from build123d import *

# Parameters (mm, degrees)
SKETCH_1_R             = 56
SKETCH_1_R_2           = 47.5
EXTRUDE_1_DEPTH        = 10
HOLE_WIZARD_M4_1_D     = 3.3
HOLE_WIZARD_M4_1_DEPTH = 7.5
CHAMFER_1_SIZE         = 0.25
SKETCH_5_R             = 50
SKETCH_5_R_2           = 48.5
CUT_EXTRUDE_1_DEPTH    = 1.2


with BuildPart() as part:
    # 草图1 → 凸台-拉伸1 (new body)
    with BuildSketch(Plane.XY):
        Circle(SKETCH_1_R)
        Circle(SKETCH_1_R_2, mode=Mode.SUBTRACT)
    extrude(amount=EXTRUDE_1_DEPTH)

    # M4 螺纹孔1
    with Locations(Plane(origin=(0, 0, 0), x_dir=(-1, 0, 0), z_dir=(0, 0, -1))):
        with Locations((35.5, 0), (0, 35.5), (0, -35.5), (-35.5, 0), (-37.476659403, -37.476659403), (37.476659403, -37.476659403), (37.476659403, 37.476659403), (-37.476659403, 37.476659403), (0, 53), (53, 0), (0, -53), (-53, 0)):
            Hole(HOLE_WIZARD_M4_1_D / 2, depth=HOLE_WIZARD_M4_1_DEPTH)

    # 倒角1
    chamfer_1_edges = [part.edges().sort_by_distance(p)[0] for p in [
        (-56, 0, 0),
        (-56, 0, 10),
        (-47.5, 0, 0),
        (-47.5, 0, 10),
    ]]
    chamfer(chamfer_1_edges, length=CHAMFER_1_SIZE)

    # 草图5 → 切除-拉伸1 (cut)
    with BuildSketch(Plane(origin=(0, 0, 0), x_dir=(-1, 0, 0), z_dir=(0, 0, -1))):
        Circle(SKETCH_5_R)
        Circle(SKETCH_5_R_2, mode=Mode.SUBTRACT)
    extrude(amount=-CUT_EXTRUDE_1_DEPTH, mode=Mode.SUBTRACT)


solid = part.part
CAD build for the part. Positions are in the model's coordinates, mm. A direction names the side the tool comes from. Round coordinates to 2 decimals unless told otherwise and drop trailing zeros. Write item = value, one per line. Start each with the question number.
(1) Probe line 1 (Y direction, x = 0, z = 3.75); line 2 (X direction, y = -0.5, z = 5.25); line 3 (X direction, y = 25.5, z = 1). List the from-to ranges inside material, lowest first. Write a range as [from, to].
(2) Which spindle directions (+Z, -Z, +X, -X, +Y, -Y) get a long thin tool onto all of the face, cutting with end or side? Do faces 3 (the cylindrical face through (-22.38, -43.028, 0.592)), 4 (the cylindrical face through (-10.3, -46.37, 4.93)). Say none if no direction does.
(3) Pin check, flat tips, straight feed: P1, Ø1, axis at x = 0.5, y = 53, coming from the -Z side; P2, Ø3, axis at x = 12.5, z = 7, coming from the -Y side; P3, Ø3, axis at y = -30.5, z = 9, coming from the +X side. Stop position of each tip, or through.
(4) Cut at C-C, the plane z = 5. State how many separate pieces and enclosed holes the cut face has, then the cut area to 3 significant figures.
(5) Pull direction X, two halves, no side cores. Call faces 1 (the cylindrical face through (38.24, -38.94, 3.8)), 2 (the flat face through (-50, 4, 0)): released by +X, released by -X, zero draft, split by the parting line, or undercut.
Model answer:
q1.line_1 = [-56, -54.65], [-51.35, -47.5], [47.5, 51.35], [54.65, 56]
q1.line_2 = [-56, -54.57], [-51.43, -47.5], [47.5, 51.43], [54.57, 56]
q1.line_3 = [-49.86, -43.01], [-41.26, -40.07], [40.07, 41.26], [43.01, 49.86]
q2.face_3 = -Z
q2.face_4 = +Z, -Z
q3.P1 = 7.5
q3.P2 = -54.91
q3.P3 = 47.91
q4.separate_pieces = 1
q4.enclosed_holes = 9
q4.area = 2,700 mm2
q5.face_1 = undercut
q5.face_2 = zero draft
